```python
from build123d import *

# Parameters (mm, degrees)
SKETCH_1_W          = 27
SKETCH_1_H          = 80
EXTRUDE_2_DEPTH     = 3
SKETCH_2_R          = 1
CUT_EXTRUDE_1_DEPTH = 15


with BuildPart() as part:
    # 草图1 → 凸台-拉伸2 (new body)
    with BuildSketch(Plane.XY):
        with Locations((-21.456521739, -18.02173913)):
            Rectangle(SKETCH_1_W, SKETCH_1_H)
    extrude(amount=EXTRUDE_2_DEPTH)

    # 草图2 → 切除-拉伸1 (cut)
    with BuildSketch(Plane(origin=(820.104098161, -68.02173913, 1111.231170435), x_dir=(-0.9925461516413246, -2.2389179114641602e-14, -0.12186934340512692), z_dir=(0, -1, 0))):
        with Locations(Location((963.085867609, 999.8129825, 0), (0, 0, 83))):
            Circle(SKETCH_2_R)
        with Locations(Location((977.974059883, 997.984942349, 0), (0, 0, 83))):
            Circle(SKETCH_2_R)
        with Locations((961.501566145, 986.909882529)):
            Circle(SKETCH_2_R)
        with Locations((976.389758419, 985.081842378)):
            Circle(SKETCH_2_R)
    extrude(amount=-CUT_EXTRUDE_1_DEPTH, mode=Mode.SUBTRACT)


solid = part.part
```
Read the model definition and answer for the solid it produces. Units are mm, in the model's axes. A direction names the side the tool comes from. Round coordinates to 2 decimals unless told otherwise and drop trailing zeros. One line per item, written item: value.
1) Consider L1, parallel to X at y = -56.1, z = 1.5. Determine where the line is inside the solid, lowest interval first. Write a range as [from, to].
Answer list:
L1: x = [-34.96, -29.96], [-27.96, -14.96], [-12.96, -7.96]
2) For faces 4 (the face through (-29.844, -55.557, 1.039)), 5 (the face through (-22, 21.978, 1)), determine the directions among +Z, -Z, +X, -X, +Y, -Y from which every point of the face is accessible in a straight line to the end or side of a thin tool.
Answer list:
face 4: -Y
face 5: +Z, -Z, +X, -X, +Y
3) Flat-ended cylindrical pins translate along their axes: P1, Ø1.6, axis at x = -28.96, z = 1.5, coming from the -Y side; P2, Ø12, axis at x = -28, y = -14, coming from the -Z side. Find the tip coordinate at first contact, or state that the pin passes through.
Answer list:
P1: stops at y = -53.02
P2: stops at z = 0
4) The mould has two halves that part along X. Classify faces 1 (the face through (-22, -17, 0)), 2 (the face through (-7.957, -19, 1)), 3 (the face through (-12.965, -55.557, 1.63)): pulls with the +X half, pulls with the -X half, needs draft (parallel to the pull), parting line crosses it, or undercut.
Answer list:
face 1: needs draft
face 2: pulls with the +X half
face 3: undercut
